Could you check a few things on this model? Use its own coordinates, in mm. A direction names the side the tool comes from. Give positions to 0.01 mm unless a question says otherwise; leave off trailing zeros. Loops run counter-clockwise (first coordinate to the right, second up) from the corner with the lowest first, then second, coordinate; pieces in that order, holes last. Notation, with made-up numbers: (49.25, 38.25) -> (88.25, 38.25) arc R20 ccw to (88.25, 67.25) -> close; hole circle Ø6 at (64, -2.75). An arc over 180 degrees is marked (long way). Put each result on its own line as item: value.
```python
from build123d import *

# Parameters (mm, degrees)
FILLET1_R = 1


with BuildPart() as part:
    # Sketch1 → Revolve1 (revolve)
    with BuildSketch(Plane.XY):
        Polygon((-54.569644219, 7.757293726), (-54.569644219, 11.770249221), (33.930355781, 11.770249221), (33.930355781, 10.770249221), (41.930355781, 10.770249221), (41.930355781, 11.770249221), (60.430355781, 11.770249221), (60.430355781, 7.770249221), (54.430355781, 7.770249221), (54.430355781, 6.770249221), (-48.569644219, 6.770249221), (-48.569644219, 7.757293726), align=None)
    revolve(axis=Axis((54.430355781, -3.229750779, 0), (-1, 0, 0)))

    # Fillet1
    fillet1_edges = [part.edges().sort_by_distance(p)[0] for p in [
        (-54.569644219, -18.229750779, 0),
        (-54.569644219, -14.216795283, 0),
        (60.430355781, -14.229750779, 0),
    ]]
    fillet(fillet1_edges, radius=FILLET1_R)


solid = part.part
```
1. I'm going to push flat-ended pins straight in: pin 1 (12 mm diameter, centred on x = -16, y = 6.5, fed in from -Z); pin 2 (10 mm diameter, centred on x = 13.5, y = -10, fed in from -Z); pin 3 (12 mm diameter, centred on x = 41.5, z = 8.5, fed in from -Y); pin 4 (12 mm diameter, centred on x = -23.5, z = -0.5, fed in from +Y). Where does each tip first touch, or does it pass through?
Recorded:
pin 1: stops at z = -14.53
pin 2: stops at z = -14.9
pin 3: stops at y = -18.02
pin 4: stops at y = 11.77
2. If we section it at B-B (x = 6): List the corners of the cut face in (y, z) for me, then the cut area to 3 significant figures.
Recorded:
outline: circle Ø30 at (-3.23, 0); hole circle Ø20 at (-3.23, 0)
area: 393 mm^2
3. For faces 1 (the face through (-48.57, -6, 10)), 2 (the face through (60.43, -10, -10.1)), 3 (the face through (33.93, -16, -7)), 4 (the face through (-9.207, -18.215, -0.66)), 5 (the face through (56.895, 1.846, 9.759)), which set-ups out of +Z, -Z, +X, -X, +Y, -Y let a thin tool reach every point of the face, with its end or its side?
Recorded:
face 1: -X
face 2: +Z, -Z, +X, +Y, -Y
face 3: none
face 4: +X, -X
face 5: +X
4. Thinking about a two-plate mould opening in Y: for faces 6 (the face through (37.986, 10.124, -4.205)), 7 (the face through (-51.1, 6.92, 4.21)), 8 (the face through (-54.57, -14, -6)), which applies, pulls with the +Y half, pulls with the -Y half, needs draft (parallel to the pull), parting line crosses it, or undercut?
Recorded:
face 6: parting line crosses it
face 7: undercut
face 8: needs draft
5. I need wall thicknesses on line 1 (Y direction, x = 58.3, z = 0); line 2 (Y direction, x = -0.5, z = 0); line 3 (Z direction, x = -44, y = -0.5). Which ranges of each line are inside material? Lowest first, please.
Recorded:
line 1: y = -18.23 to -14.23, 7.77 to 11.77
line 2: y = -18.23 to -13.23, 6.77 to 11.77
line 3: z = -14.75 to -9.62, 9.62 to 14.75
